Check sheet for the modelled part. Datum: model origin and axes. Units: mm. Face numbers are marked on the shaded views. A direction names the side the tool comes from. Give positions to 0.01 mm unless a question says otherwise; leave off trailing zeros. Loops run counter-clockwise (first coordinate to the right, second up) from the corner with the lowest first, then second, coordinate; pieces in that order, holes last.
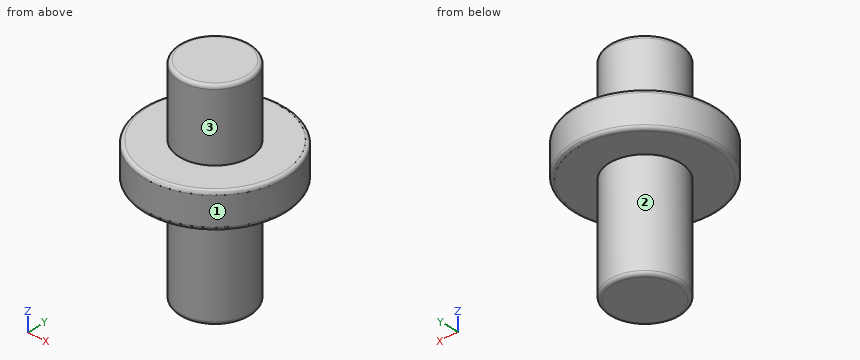
```python
from build123d import *

# Parameters (mm, degrees)
SKETCH_1_R      = 2
EXTRUDE_1_DEPTH = 6
SKETCH_2_R      = 4
EXTRUDE_2_DEPTH = 2
SKETCH_3_R      = 2
EXTRUDE_3_DEPTH = 4
FILLET_1_R      = 0.2
FILLET_2_R      = 0.2


with BuildPart() as part:
    # 草图1 → 凸台-拉伸1 (new body)
    with BuildSketch(Plane.XY):
        Circle(SKETCH_1_R)
    extrude(amount=EXTRUDE_1_DEPTH)

    # 草图2 → 凸台-拉伸2 (add)
    with BuildSketch(Plane.XY.offset(6)):
        Circle(SKETCH_2_R)
    extrude(amount=EXTRUDE_2_DEPTH)

    # 草图3 → 凸台-拉伸3 (add)
    with BuildSketch(Plane.XY.offset(8)):
        Circle(SKETCH_3_R)
    extrude(amount=EXTRUDE_3_DEPTH)

    # 圆角1
    fillet_1_edges = [part.edges().sort_by_distance(p)[0] for p in [
        (-2, 0, 12),
        (-2, 0, 0),
    ]]
    fillet(fillet_1_edges, radius=FILLET_1_R)

    # 圆角2
    fillet_2_edges = [part.edges().sort_by_distance(p)[0] for p in [
        (-4, 0, 6),
        (-4, 0, 8),
    ]]
    fillet(fillet_2_edges, radius=FILLET_2_R)


solid = part.part
```
(1) Section check C-C on z = 3.5. Record the boundary of the cut face in (x, y), plus the area to 3 significant figures.
(2) Access from +Z, -Z, +X, -X, +Y, -Y to the whole of each face (thin tool, end or side, straight path). Record for the marked faces 1, 2 and 3.
(3) Section check D-D on z = 7.5. Record the boundary of the cut face in (x, y).
(4) Gauge pin test, flat ends, axial feed: pin 1 Ø3 at (x, y) = (0.5, -3) entering from -Z; pin 2 Ø4 at (y, z) = (-0.5, 2.5) entering from -X; pin 3 Ø3 at (x, z) = (-3, 3.5) entering from +Y; pin 4 Ø1.5 at (y, z) = (2.5, 2.5) entering from +X. Record the tip position at first contact, or that the pin passes through.
(5) Section check A-A on y = 0. Record the boundary of the cut face in (x, z).
(6) Material ranges on line 1 (Z direction, x = -1.5, y = -1.5); line 2 (X direction, y = -0.25, z = 1.25); line 3 (X direction, y = 2.75, z = 6.25), recorded low to high.
Computed values:
1. outline: circle Ø4 at (0, 0)
1. area: 12.6 mm2
2. face 1: +Z, -Z
2. face 2: -Z
2. face 3: +Z
3. outline: circle Ø8 at (0, 0)
4. pin 1: stops at z = 0
4. pin 2: stops at x = -2
4. pin 3: stops at y = 1.32
4. pin 4: stops at x = 0.97
5. outline: (-4, 6.2) arc R0.2 ccw to (-3.8, 6) - (-2, 6) - (-2, 0.2) arc R0.2 ccw to (-1.8, 0) - (1.8, 0) arc R0.2 ccw to (2, 0.2) - (2, 6) - (3.8, 6) arc R0.2 ccw to (4, 6.2) - (4, 7.8) arc R0.2 ccw to (3.8, 8) - (2, 8) - (2, 11.8) arc R0.2 ccw to (1.8, 12) - (-1.8, 12) arc R0.2 ccw to (-2, 11.8) - (-2, 8) - (-3.8, 8) arc R0.2 ccw to (-4, 7.8) - close
6. line 1: z = 6 to 8
6. line 2: x = -1.98 to 1.98
6. line 3: x = -2.9 to 2.9
